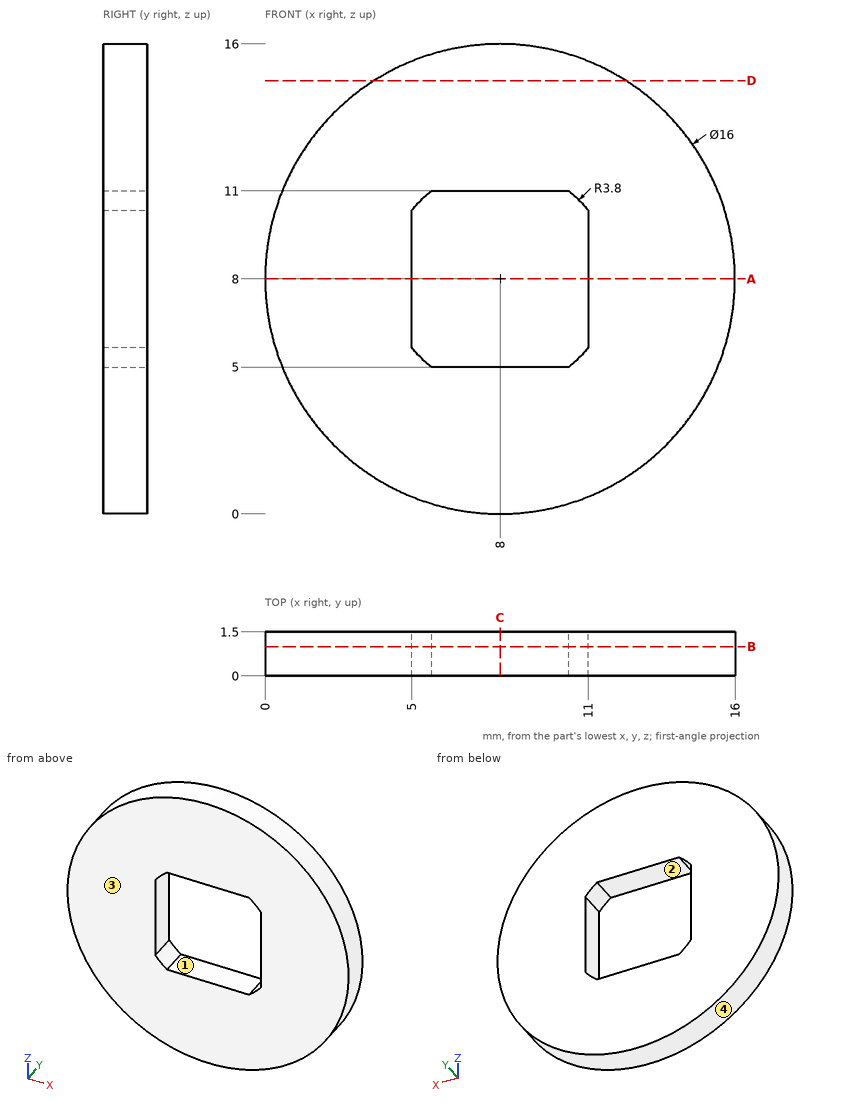
Could you check a few things on this drawing? It's one solid part, dimensions in mm from its lowest x, y, z. Round coordinates to 2 decimals unless told otherwise and drop trailing zeros. Write each loop counter-clockwise with the first axis right and the second up, starting at its lowest first coordinate (ties: lowest second). Pieces come first, ordered by that corner, then holes. Notation, with made-up numbers: (73, 0) -> (84, 0) arc R18 cw to (84, 7) -> close; hole circle Ø10 at (-7, -13.5). An arc over 180 degrees is marked (long way). One line per question, with ' | ' between items. Start each with the question number.
1) I need wall thicknesses on line 1 (X direction, y = 0.9, z = 8); line 2 (X direction, y = 0.7, z = 9.25). Which ranges of each line are inside material? Lowest first, please. Write a range as [from, to].
2) If we mould it in two halves opening along Z, with no side actions, what happens to the marked faces 1, 2, 3 and 4? For each: released by +Z, released by -Z, zero draft, split by the parting line, or undercut.
3) Suppose I cut it at A-A on z = 8. Write out the boundary of the cut face in (x, y), then the cut area to 3 significant figures.
4) Suppose I cut it at C-C on x = 8. Write out the boundary of the cut face in (y, z), then the cut area to 3 significant figures.
5) Suppose I cut it at B-B on y = 1. Write out the boundary of the cut face in (x, z), then the cut area to 3 significant figures.
6) Suppose I cut it at D-D on z = 14.75. Write out the boundary of the cut face in (x, y).
Return value:
1) line 1: x = [0, 5], [11, 16] | line 2: x = [0.1, 5], [11, 15.9]
2) face 1: undercut | face 2: undercut | face 3: zero draft | face 4: split by the parting line
3) outline: (0, 0) -> (5, 0) -> (5, 1.5) -> (0, 1.5) -> close; (11, 0) -> (16, 0) -> (16, 1.5) -> (11, 1.5) -> close | area: 15.0 mm2
4) outline: (0, 0) -> (1.5, 0) -> (1.5, 5) -> (0, 5) -> close; (0, 11) -> (1.5, 11) -> (1.5, 16) -> (0, 16) -> close | area: 15.0 mm2
5) outline: circle Ø16 at (8, 8); hole (5, 5.67) arc R3.8 ccw to (5.67, 5) -> (10.33, 5) arc R3.8 ccw to (11, 5.67) -> (11, 10.33) arc R3.8 ccw to (10.33, 11) -> (5.67, 11) arc R3.8 ccw to (5, 10.33) -> close | area: 166 mm2
6) outline: (3.71, 0) -> (12.29, 0) -> (12.29, 1.5) -> (3.71, 1.5) -> close
